Verification items for the finished model (mm, model axes). A direction names the side the tool comes from. Round coordinates to 2 decimals unless told otherwise and drop trailing zeros. Write each loop counter-clockwise with the first axis right and the second up, starting at its lowest first coordinate (ties: lowest second). Pieces come first, ordered by that corner, then holes. Notation, with made-up numbers: (6, 69) - (39, 69) arc R18 cw to (39, 80) - close; hole circle Ø5 at (65, 53.25). An arc over 180 degrees is marked (long way). Answer as a JSON object with one key per item and string values.
```python
from build123d import *

# Parameters (mm, degrees)
EXTRUDE_387_DEPTH = 7.5
FILLET_1280_R     = 0.6


with BuildPart() as part:
    # 草图1 → Extrude 387 (new body)
    with BuildSketch(Plane(origin=(0, 0, 0), x_dir=(0, 0, -1), z_dir=(1, 0, 0))):
        Polygon((9, 5.196152423), (9, -5.196152423), (0, -10.392304845), (-9, -5.196152423), (-9, 5.196152423), (0, 10.392304845), align=None)
    extrude(amount=EXTRUDE_387_DEPTH)

    # 草图2 → 凸台-旋转1 (revolve)
    with BuildSketch(Plane.XY, mode=Mode.PRIVATE) as revolve_1_sk:
        Polygon((0, 0), (57.5, 0), (57.5, 4.4845), (57.5, 6), (27.5, 6), (0, 6), align=None)
    revolve(revolve_1_sk.sketch.rotate(Axis((0, 0, 0), (1, 0, 0)), 90), axis=Axis((0, 0, 0), (1, 0, 0)))

    # 草图3 → 切除-旋转1 (revolve, cut)
    with BuildSketch(Plane.XY):
        Polygon((0, 9), (3.690598923, 15.392304845), (3.690598923, 20.392304845), (-10, 20.392304845), (-10, 9), align=None)
    revolve(axis=Axis((0, 0, 0), (1, 0, 0)), mode=Mode.SUBTRACT)

    # 草图4 → 切除-旋转3 (revolve, cut)
    with BuildSketch(Plane.XY, mode=Mode.PRIVATE) as cut_revolve_3_sk:
        Polygon((7.5, 8.315), (6.9, 8.661410162), (6.9, 10.392304845), (7.5, 10.392304845), align=None)
    revolve(cut_revolve_3_sk.sketch.rotate(Axis((0, 0, 0), (1, 0, 0)), 90), axis=Axis((0, 0, 0), (1, 0, 0)), mode=Mode.SUBTRACT)

    # Fillet 1280
    fillet_1280_edges = [part.edges().sort_by_distance(p)[0] for p in [
        (7.5, 0, -6),
    ]]
    fillet(fillet_1280_edges, radius=FILLET_1280_R)


solid = part.part
```
Q1. Section check A-A, the plane x = 46.5. Record the cut outline in (y, z), then the cut area to 3 significant figures.
Geometry check:
{"outline": "circle Ø12 at (0, 0)", "area": "113 mm2"}
Q2. Set-up check for faces 1 (the cylindrical face through (32.454, -1.802, 5.723)), 2 (the conical face through (0.2, 4.69, 8.08)): record each of +Z, -Z, +X, -X, +Y, -Y from which the full face is reachable in a straight line by a thin tool's end or side.
Geometry check:
{"face 1": "+X", "face 2": "+Z, -X, +Y"}
Q3. Material ranges on line 1 along X through (y, z) = (4, 5.25); line 2 along Z through (x, y) = (14, -0.25); line 3 along Y through (x, z) = (5.5, 4.5), recorded low to high. Write a range as [from, to].
Geometry check:
{"line 1": "x = [0, 7.5]", "line 2": "z = [-5.99, 5.99]", "line 3": "y = [-7.79, 7.79]"}
Q4. Gauge pin test, flat ends, axial feed: P1, Ø8, axis at x = 44.5, z = 2, coming from the +Y side; P2, Ø4, axis at x = 44.5, y = -2.5, coming from the +Z side; P3, Ø5, axis at x = 51, y = 1, coming from the -Z side. Record the tip position at first contact, or that the pin passes through.
Geometry check:
{"P1": "stops at y = 6", "P2": "stops at z = 5.98", "P3": "stops at z = -6"}
